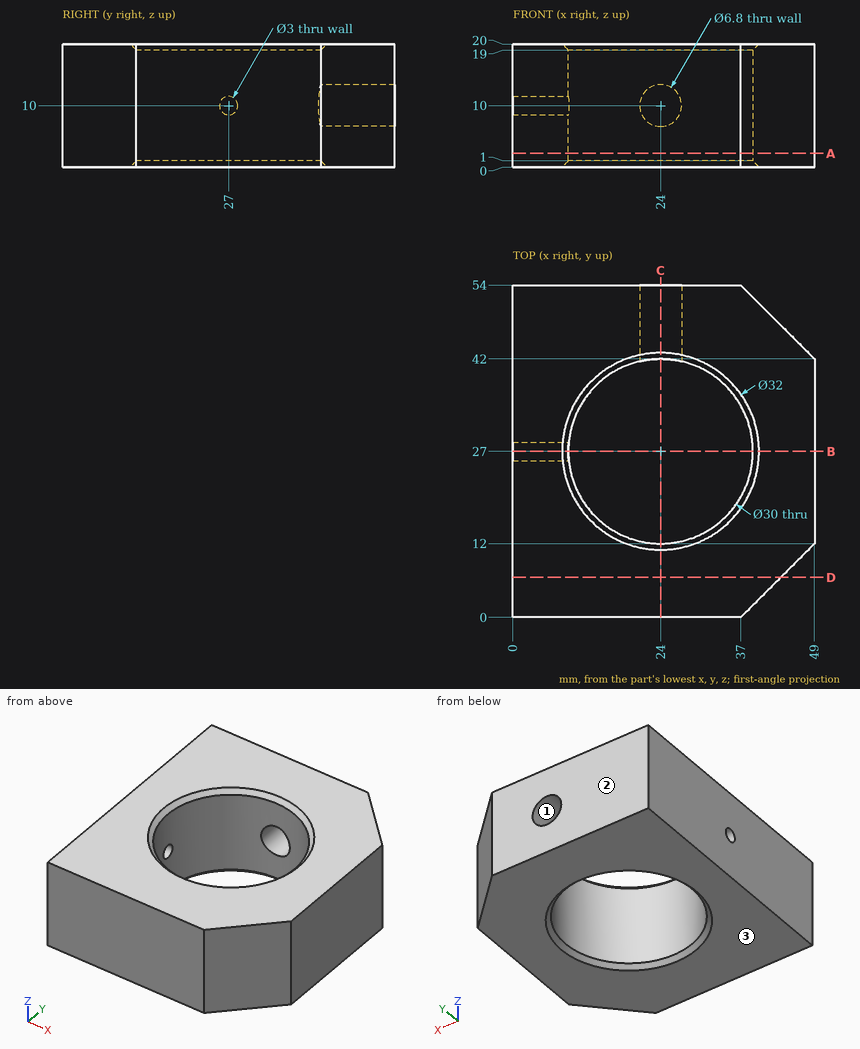
Can you work these out from the drawing? Everything is in mm from the part's minimum corner. Round coordinates to 2 decimals unless told otherwise and drop trailing zeros. Loops run counter-clockwise (first coordinate to the right, second up) from the corner with the lowest first, then second, coordinate; pieces in that order, holes last. Notation, with made-up numbers: (87, 24) - (94, 24) arc R5 ccw to (94, 29) - close; hole circle Ø4 at (82, 11). An arc over 180 degrees is marked (long way). Answer in a Markdown table with one row per item. Add a question column.
Q1. I want a section at D-D on y = 6.5. List the corners of the cut face in (x, z) for me, and give its area (3 significant figures).
Q2. I want a section at B-B on y = 27. List the corners of the cut face in (x, z) for me, and give its area (3 significant figures).
Q3. I need wall thicknesses on L1, parallel to X at y = 27, z = 14; L2, parallel to Y at x = 5.25, z = 10; L3, parallel to X at y = 32, z = 9.5. Which ranges of each line are inside material? Lowest first, please.
Q4. For pin 1 Ø3 at (x, y) = (20, 13.5) entering from -Z, with a flat end and sliding along its axis, tell me the tip position at first contact or that it passes through.
Q5. I want a section at C-C on x = 24. List the corners of the cut face in (y, z) for me, and give its area (3 significant figures).
Q6. I want a section at A-A on z = 2.25. List the corners of the cut face in (x, y) for me.
Q7. We'd pull the mould along Z, two halves only. Please class the marked faces 1, 2 and 3: pulls with the +Z half, pulls with the -Z half, needs draft (parallel to the pull), parting line crosses it, or undercut.
A:
| question | item | result |
|---|---|---|
| 1 | outline | (0, 0) - (43.5, 0) - (43.5, 20) - (0, 20) - close |
| 1 | area | 870 mm^2 |
| 2 | outline | (0, 0) - (8, 0) - (9, 1) - (9, 8.5) - (0, 8.5) - close; (0, 11.5) - (9, 11.5) - (9, 19) - (8, 20) - (0, 20) - close; (39, 1) - (40, 0) - (49, 0) - (49, 20) - (40, 20) - (39, 19) - close |
| 2 | area | 351 mm^2 |
| 3 | L1 | 0 to 9, 39 to 49 |
| 3 | L2 | 0 to 25.5, 28.5 to 54 |
| 3 | L3 | 0 to 9.86, 38.14 to 49 |
| 4 | pin 1 | z = 0.42 |
| 5 | outline | (0, 0) - (11, 0) - (12, 1) - (12, 19) - (11, 20) - (0, 20) - close; (42, 1) - (43, 0) - (54, 0) - (54, 6.6) - (42, 6.6) - close; (42, 13.4) - (54, 13.4) - (54, 20) - (43, 20) - (42, 19) - close |
| 5 | area | 396 mm^2 |
| 6 | outline | (0, 0) - (37, 0) - (49, 12) - (49, 42) - (37, 54) - (0, 54) - close; hole circle Ø30 at (24, 27) |
| 7 | face 1 | undercut |
| 7 | face 2 | needs draft |
| 7 | face 3 | pulls with the -Z half |
